For this review, use the dimensioned drawing (mm, ordinates from the lowest corner) and the shaded views. A direction names the side the tool comes from. Coordinates: 2 decimals unless noted, no trailing zeros. Loops run counter-clockwise (first coordinate to the right, second up) from the corner with the lowest first, then second, coordinate; pieces in that order, holes last. Notation, with made-up numbers: (75, -0.5) - (79, -0.5) arc R30 ccw to (79, 30.5) - close; hole circle Ø5 at (8.5, 2.25). An arc over 180 degrees is marked (long way). Answer in a Markdown table with one row per item. Add a question column.
(1) Clearance check with flat-ended pins moving along their axes: pin 1 (4.5 mm diameter, centred on x = 19, y = 10, fed in from +Z); pin 2 (8 mm diameter, centred on x = 18.5, y = 9.5, fed in from +Z); pin 3 (3 mm diameter, centred on x = 6, y = 48.5, fed in from -Z). State where each tip first meets the part, or that it passes through.
(2) We need section A-A, the plane x = 6. Write out the cut boundary in (y, z), plus the area to 3 significant figures.
(3) We need section B-B, the plane y = 10. Write out the cut boundary in (x, z), plus the area to 3 significant figures.
(4) To check wall thickness, follow L1, parallel to Y at x = 19, z = 4.5; L2, parallel to Y at x = 6, z = 2.05; L3, parallel to X at y = 12.5, z = 5.5. State the ranges of each line that lie inside material, in increasing order. Write a range as [from, to].
(5) For the marked faces 5, 6 and 7, list the 3-axis set-ups (+Z, -Z, +X, -X, +Y, -Y) from which the entire face can be reached by the end or side of a thin tool; tool diameter is ignored.
(6) The part is to be moulded in two halves that separate along Y. For the marked faces 1, 2, 3 and 4, say which applies: released by +Y, released by -Y, zero draft, split by the parting line, or undercut.
(7) We need section C-C, the plane z = 9.5. Write out the cut boundary in (x, y).
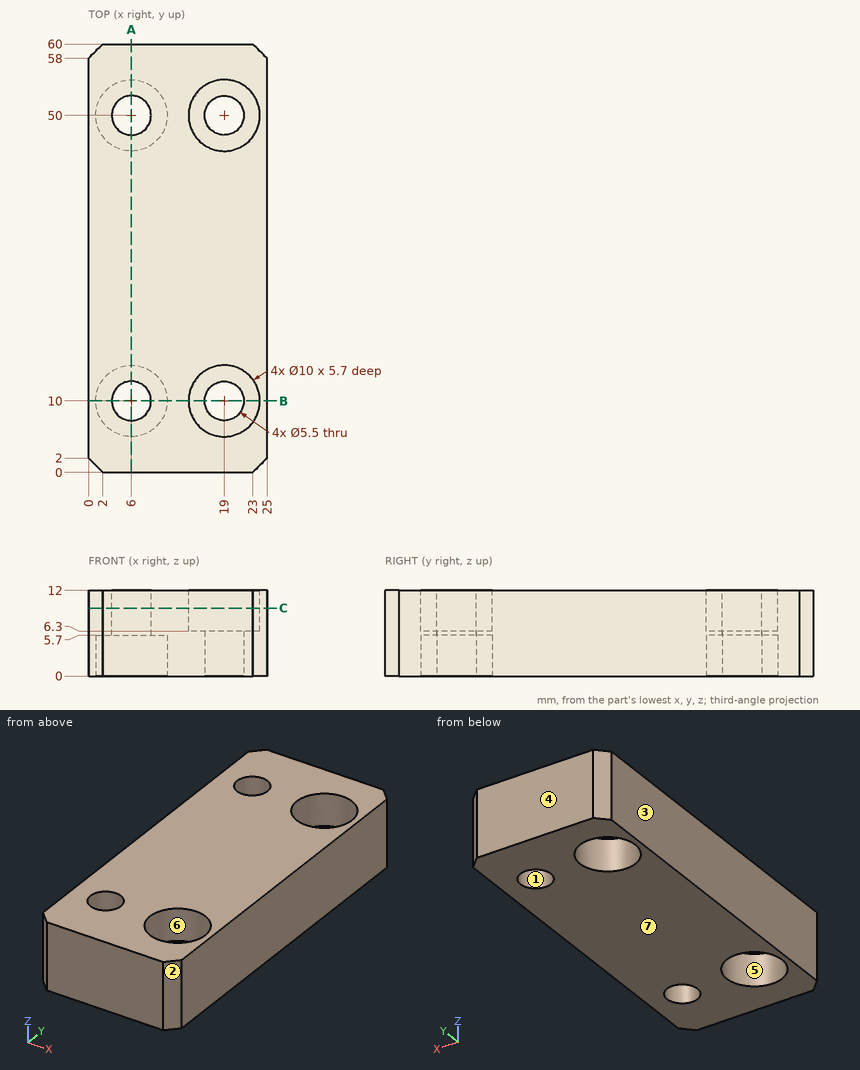
Responses:
| question | item | result |
|---|---|---|
| 1 | pin 1 | passes through |
| 1 | pin 2 | stops at z = 6.3 |
| 1 | pin 3 | stops at z = 5.7 |
| 2 | outline | (0, 0) - (5, 0) - (5, 5.7) - (7.25, 5.7) - (7.25, 12) - (0, 12) - close; (12.75, 5.7) - (15, 5.7) - (15, 0) - (45, 0) - (45, 5.7) - (47.25, 5.7) - (47.25, 12) - (12.75, 12) - close; (52.75, 5.7) - (55, 5.7) - (55, 0) - (60, 0) - (60, 12) - (52.75, 12) - close |
| 2 | area | 537 mm2 |
| 3 | outline | (0, 0) - (1, 0) - (1, 5.7) - (3.25, 5.7) - (3.25, 12) - (0, 12) - close; (8.75, 5.7) - (11, 5.7) - (11, 0) - (16.25, 0) - (16.25, 6.3) - (14, 6.3) - (14, 12) - (8.75, 12) - close; (21.75, 0) - (25, 0) - (25, 12) - (24, 12) - (24, 6.3) - (21.75, 6.3) - close |
| 3 | area | 117 mm2 |
| 4 | L1 | y = [0, 7.25], [12.75, 47.25], [52.75, 60] |
| 4 | L2 | y = [0, 5], [15, 45], [55, 60] |
| 4 | L3 | x = [0, 1.67], [10.33, 17.85], [20.15, 25] |
| 5 | face 5 | -Z |
| 5 | face 6 | +Z |
| 5 | face 7 | -Z, +X, -X, +Y, -Y |
| 6 | face 1 | undercut |
| 6 | face 2 | released by -Y |
| 6 | face 3 | zero draft |
| 6 | face 4 | released by +Y |
| 7 | outline | (0, 2) - (2, 0) - (23, 0) - (25, 2) - (25, 58) - (23, 60) - (2, 60) - (0, 58) - close; hole circle Ø5.5 at (6, 10); hole circle Ø5.5 at (6, 50); hole circle Ø10 at (19, 10); hole circle Ø10 at (19, 50) |
